Input: part model. Units: mm. Frame: model coordinates. A direction names the side the tool comes from. Give positions to 0.01 mm unless a question says otherwise; leave off trailing zeros. Loops run counter-clockwise (first coordinate to the right, second up) from the corner with the lowest first, then second, coordinate; pieces in that order, holes last. Notation, with made-up numbers: M 64.5,87 L 102.5,87 A20 ccw 102.5,125 Z; hole C -24,-30 d5. An arc over 180 degrees is marked long. Answer as a JSON object with one key per item and string values. Group by question number.
1) First-contact query: P1, Ø0.8, axis at x = 15, y = 3.5, coming from the +Z side; P2, Ø1.3, axis at y = 3.66, z = 5.51, coming from the -X side. Flat tips, straight axial feed; report the tip coordinate or a pass-through.
2) Draft query along Z for faces 1 (the cylindrical face through (-13.97, 2.22, -0.41)), 2 (the flat face through (14, 2.75, -4)), 3 (the cylindrical face through (0.14, 0.6, -8.43)), 4 (the flat face through (12, 3, 4)). Return one class per face: +Z half, -Z half, draft (parallel to the pull), parting line (faces both ways), or undercut.
3) Section query A-A on x = 13. Return loops of the section in (y, z), plus the area to 3 significant figures.
4) Section query C-C on x = 7.5. Return loops of the section in (y, z).
5) Section query B-B on y = 0.5. Return loops of the section in (x, z), plus the area to 3 significant figures.
6) Ray query, L1, parallel to Y at x = -14.95, z = 0; L2, parallel to Z at x = 12.5, y = 2.5; L3, parallel to X at y = 3, z = 0.75. Return the intervals inside material, ascending.
7) Access query for faces 5 (the cylindrical face through (11.43, 0.6, 0.1)), 6 (the flat face through (-12, 4, 6)), 7 (the flat face through (-12, 4.7, 6.8)), 8 (the cylindrical face through (13.97, 4.24, 2.2)). Directions: +Z, -Z, +X, -X, +Y, -Y. A direction counts if a zero-diameter tool reaches every point of the face in a straight line with its end or side. Return the directions, or none.
from build123d import *

# Parameters (mm, degrees)
HOUSING_BODY_DEPTH               = 7
HOUSING_EDGE_FILLET_R2_R         = 2
PIN_SET_A_SKETCH_R               = 1.5
PIN_SET_A_SKETCH_R_2             = 1.1
TUBULAR_PINS_SET_A_3_DEPTH       = 4
PIN_SET_B_AND_TAB_SKETCH_R       = 1.5
PIN_SET_B_AND_TAB_SKETCH_R_2     = 1.1
PIN_SET_B_AND_TAB_SKETCH_W       = 4.5
PIN_SET_B_AND_TAB_SKETCH_H       = 1.5
TUBULAR_PINS_SET_B_AND_TAB_DEPTH = 4


with BuildPart() as part:
    # Housing Profile Sketch → Housing Body (new body)
    with BuildSketch(Plane(origin=(0, 0, 0), x_dir=(1, 0, 0), z_dir=(0, 1, 0))):
        with BuildLine():
            Line((-10, 9), (10, 9))
            ThreePointArc((10, 9), (11.414213562, 8.414213562), (12, 7))
            Line((12, 7), (12, -7))
            ThreePointArc((12, -7), (11.414213562, -8.414213562), (10, -9))
            Line((10, -9), (-10, -9))
            ThreePointArc((-10, -9), (-11.414213562, -8.414213562), (-12, -7))
            Line((-12, -7), (-12, 7))
            ThreePointArc((-12, 7), (-11.414213562, 8.414213562), (-10, 9))
        make_face()
    extrude(amount=HOUSING_BODY_DEPTH)

    # Housing Edge Fillet R2
    housing_edge_fillet_r2_edges = [part.edges().sort_by_distance(p)[0] for p in [
        (-12, 0, 0),
        (-11.414213562, 0, -8.414213562),
        (0, 0, -9),
        (11.414213562, 0, -8.414213562),
        (-11.414213562, 7, -8.414213562),
        (-12, 7, 0),
        (-11.414213562, 7, 8.414213562),
        (0, 7, 9),
        (11.414213562, 7, 8.414213562),
        (12, 7, 0),
        (11.414213562, 7, -8.414213562),
        (12, 0, 0),
        (0, 7, -9),
        (11.414213562, 0, 8.414213562),
        (0, 0, 9),
        (-11.414213562, 0, 8.414213562),
    ]]
    fillet(housing_edge_fillet_r2_edges, radius=HOUSING_EDGE_FILLET_R2_R)

    # Pin Set A Sketch → Tubular Pins Set A Ø3 (add)
    # profile 1 of 3: a face of its own
    with BuildSketch(Plane.ZY.offset(12)):
        with Locations(Location((0, 3.661725767, 0), (0, 0, 116.851166023))):
            Circle(PIN_SET_A_SKETCH_R)
        with Locations((0, 3.661725767)):
            Circle(PIN_SET_A_SKETCH_R_2, mode=Mode.SUBTRACT)
    # profile 2 of 3: a face of its own
    with BuildSketch(Plane.ZY.offset(12)):
        with Locations(Location((-5.731156871, 3.661725767, 0), (0, 0, 212.232000091))):
            Circle(PIN_SET_A_SKETCH_R)
        with Locations((-5.731156871, 3.661725767)):
            Circle(PIN_SET_A_SKETCH_R_2, mode=Mode.SUBTRACT)
    # profile 3 of 3: a face of its own
    with BuildSketch(Plane.ZY.offset(12)):
        with Locations(Location((5.508783942, 3.661725767, 0), (0, 0, 116.851166023))):
            Circle(PIN_SET_A_SKETCH_R)
        with Locations((5.508783942, 3.661725767)):
            Circle(PIN_SET_A_SKETCH_R_2, mode=Mode.SUBTRACT)
    extrude(amount=TUBULAR_PINS_SET_A_3_DEPTH)

    # Pin Set B and Tab Sketch → Tubular Pins Set B and Tab (add)
    # profile 1 of 3: a face of its own
    with BuildSketch(Plane(origin=(12, 0, 0), x_dir=(0, 0, -1), z_dir=(1, 0, 0))):
        with Locations(Location((-5.785268851, 3.5, 0), (0, 0, 215.921576532))):
            Circle(PIN_SET_B_AND_TAB_SKETCH_R)
        with Locations((-5.785268851, 3.5)):
            Circle(PIN_SET_B_AND_TAB_SKETCH_R_2, mode=Mode.SUBTRACT)
    # profile 2 of 3: a face of its own
    with BuildSketch(Plane(origin=(12, 0, 0), x_dir=(0, 0, -1), z_dir=(1, 0, 0))):
        with Locations(Location((-1.385268851, 3.5, 0), (0, 0, 270))):
            Circle(PIN_SET_B_AND_TAB_SKETCH_R)
        with Locations((-1.385268851, 3.5)):
            Circle(PIN_SET_B_AND_TAB_SKETCH_R_2, mode=Mode.SUBTRACT)
    # profile 3 of 3: a face of its own
    with BuildSketch(Plane(origin=(12, 0, 0), x_dir=(0, 0, -1), z_dir=(1, 0, 0))):
        with Locations((4.21427792, 3.5)):
            Rectangle(PIN_SET_B_AND_TAB_SKETCH_W, PIN_SET_B_AND_TAB_SKETCH_H)
    extrude(amount=TUBULAR_PINS_SET_B_AND_TAB_DEPTH)


solid = part.part
Output:
{
 "1": {"P1": "stops at z = 7.29", "P2": "stops at x = -12"},
 "2": {"face 1": "undercut", "face 2": "draft", "face 3": "-Z half", "face 4": "undercut"},
 "3": {"outline": "C 3.5,1.39 d3; C 3.5,5.79 d3; M 2.75,-6.46 L 4.25,-6.46 L 4.25,-1.96 L 2.75,-1.96 Z; hole C 3.5,1.39 d2.2; hole C 3.5,5.79 d2.2", "area": "13.3 mm^2"},
 "4": {"outline": "M 0,-7 A2 ccw 2,-9 L 5,-9 A2 ccw 7,-7 L 7,7 A2 ccw 5,9 L 2,9 A2 ccw 0,7 Z"},
 "5": {"outline": "M -11.32,-7 A1.32 ccw -10,-8.32 L 10,-8.32 A1.32 ccw 11.32,-7 L 11.32,7 A1.32 ccw 10,8.32 L -10,8.32 A1.32 ccw -11.32,7 Z", "area": "375 mm^2"},
 "6": {"L1": "y = 2.16 to 2.56, 4.76 to 5.16", "L2": "z = 0.27 to 0.93, 1.84 to 2.5, 4.67 to 5.33, 6.24 to 6.9", "L3": "x = -12 to 12"},
 "7": {"face 5": "+Z, -Z, +X, -Y", "face 6": "-X", "face 7": "+Z, -X, +Y", "face 8": "+X"}
}
